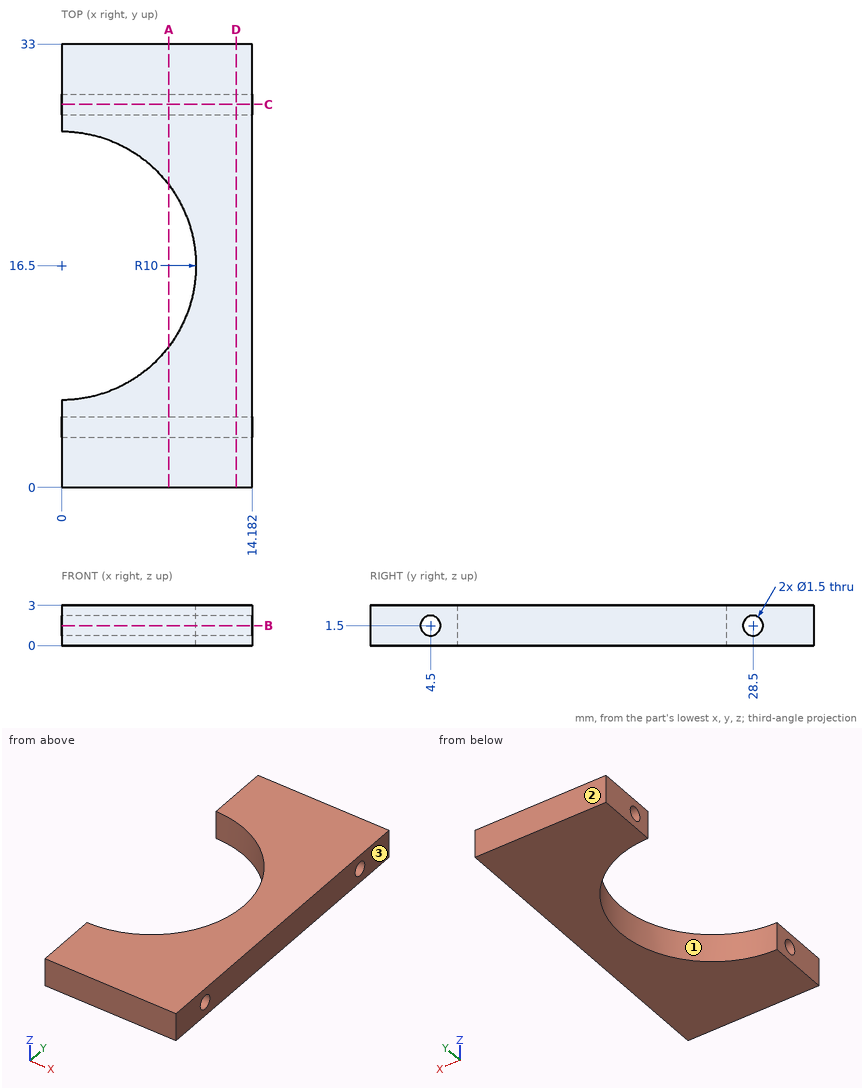
Drawing for the job (mm, zero at the part's lowest x, y, z). Coordinates: 2 decimals unless noted, no trailing zeros. Order: outer loops, then holes, each group sorted by start corner. A loop starts at its lowest first (then second) coordinate and runs counter-clockwise, first axis right, second up. Notation, with made-up numbers: (-2, 20) - (5, 20) arc R17 ccw to (5, 29) - close; hole circle Ø7 at (73, 37.5). An arc over 180 degrees is marked (long way). Use a Markdown table: item, result. Add a question column.
(1) Saw through at B-B (z = 1.5). Give the cut face in (x, y).
(2) Pull direction Y, two halves, no side cores. Call the marked faces 1, 2 and 3: +Y half, -Y half, draft (parallel to the pull), parting line (faces both ways), or undercut.
(3) Flat gauge pins, fed straight in: pin 1 (3 mm diameter, centred on x = 6.5, y = 21, fed in from -Z); pin 2 (4 mm diameter, centred on x = 9.5, y = 18.5, fed in from -Z). Where does each tip first touch, or does it go through?
(4) Saw through at A-A (x = 8). Give the cut face in (y, z).
(5) Drill centre lines: line 1 along Y through (x, z) = (10.25, 1.5); line 2 along Y through (x, z) = (4.75, 1.2); line 3 along Y through (x, z) = (2.25, 1.6). Where is each one in solid material? Low to high. Write a range as [from, to].
(6) Saw through at C-C (y = 28.5). Give the cut face in (x, z).
(7) Saw through at D-D (x = 13). Give the cut face in (y, z).
Solved:
| question | item | result |
|---|---|---|
| 1 | outline | (0, 0) - (14.18, 0) - (14.18, 3.75) - (0, 3.75) - close; (0, 5.25) - (14.18, 5.25) - (14.18, 27.75) - (0, 27.75) - (0, 26.5) arc R10 cw to (0, 6.5) - close; (0, 29.25) - (14.18, 29.25) - (14.18, 33) - (0, 33) - close |
| 2 | face 1 | undercut |
| 2 | face 2 | +Y half |
| 2 | face 3 | draft |
| 3 | pin 1 | passes through |
| 3 | pin 2 | stops at z = 0 |
| 4 | outline | (0, 0) - (10.5, 0) - (10.5, 3) - (0, 3) - close; (22.5, 0) - (33, 0) - (33, 3) - (22.5, 3) - close; hole circle Ø1.5 at (4.5, 1.5); hole circle Ø1.5 at (28.5, 1.5) |
| 5 | line 1 | y = [0, 3.75], [5.25, 27.75], [29.25, 33] |
| 5 | line 2 | y = [0, 3.81], [5.19, 7.7], [25.3, 27.81], [29.19, 33] |
| 5 | line 3 | y = [0, 3.76], [5.24, 6.76], [26.24, 27.76], [29.24, 33] |
| 6 | outline | (0, 0) - (14.18, 0) - (14.18, 0.75) - (0, 0.75) - close; (0, 2.25) - (14.18, 2.25) - (14.18, 3) - (0, 3) - close |
| 7 | outline | (0, 0) - (33, 0) - (33, 3) - (0, 3) - close; hole circle Ø1.5 at (4.5, 1.5); hole circle Ø1.5 at (28.5, 1.5) |
